Part model, mm, in its own coordinate system. Face numbers are marked on the shaded views. A direction names the side the tool comes from. Coordinates: 2 decimals unless noted, no trailing zeros. Write each loop counter-clockwise with the first axis right and the second up, starting at its lowest first coordinate (ties: lowest second). Pieces come first, ordered by that corner, then holes. Notation, with made-up numbers: (-7.5, 70) -> (22.5, 70) arc R26 cw to (22.5, 108) -> close; hole circle Ø5 at (-9.75, 38.25). An arc over 180 degrees is marked (long way). Write item = value, one per line.
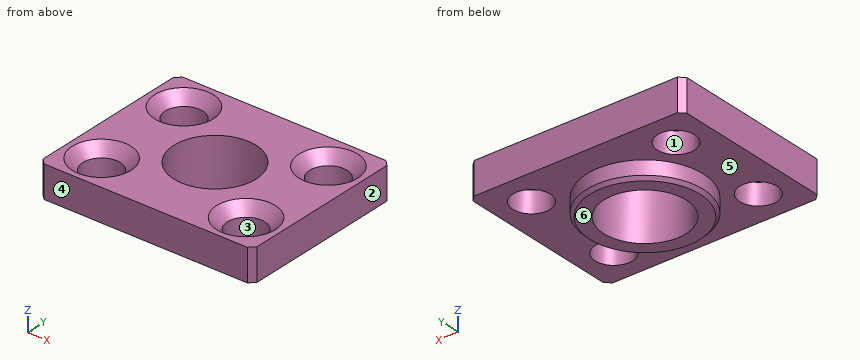
from build123d import *

# Parameters (mm, degrees)
SKETCH1_R           = 5.45
SKETCH1_R_2         = 3.85
BOSS_EXTRUDE1_DEPTH = 1.6
SKETCH2_W           = 20
SKETCH2_H           = 16
SKETCH2_R           = 3.85
SKETCH2_R_2         = 1.75
BOSS_EXTRUDE2_DEPTH = 3
CHAMFER1_SIZE       = 0.3
CHAMFER2_SIZE       = 1
CHAMFER3_SIZE       = 0.5


with BuildPart() as part:
    # Sketch1 → Boss-Extrude1 (new body)
    with BuildSketch(Plane.XY):
        Circle(SKETCH1_R)
        Circle(SKETCH1_R_2, mode=Mode.SUBTRACT)
    extrude(amount=BOSS_EXTRUDE1_DEPTH)

    # Sketch2 → Boss-Extrude2 (add)
    with BuildSketch(Plane.XY.offset(1.6)):
        Rectangle(SKETCH2_W, SKETCH2_H)
        Circle(SKETCH2_R, mode=Mode.SUBTRACT)
        with Locations((-6.75, 4.75)):
            Circle(SKETCH2_R_2, mode=Mode.SUBTRACT)
        with Locations((-6.75, -4.75)):
            Circle(SKETCH2_R_2, mode=Mode.SUBTRACT)
        with Locations((6.75, -4.75)):
            Circle(SKETCH2_R_2, mode=Mode.SUBTRACT)
        with Locations((6.75, 4.75)):
            Circle(SKETCH2_R_2, mode=Mode.SUBTRACT)
    extrude(amount=BOSS_EXTRUDE2_DEPTH)

    # Chamfer1
    chamfer1_edges = [part.edges().sort_by_distance(p)[0] for p in [
        (-5.45, 0, 0),
    ]]
    chamfer(chamfer1_edges, length=CHAMFER1_SIZE)

    # Chamfer2
    chamfer2_edges = [part.edges().sort_by_distance(p)[0] for p in [
        (-8.5, 4.75, 4.6),
        (-8.5, -4.75, 4.6),
        (5, -4.75, 4.6),
        (5, 4.75, 4.6),
    ]]
    chamfer(chamfer2_edges, length=CHAMFER2_SIZE)

    # Chamfer3
    chamfer3_edges = [part.edges().sort_by_distance(p)[0] for p in [
        (10, -8, 3.1),
        (10, 8, 3.1),
        (-10, 8, 3.1),
        (-10, -8, 3.1),
    ]]
    chamfer(chamfer3_edges, length=CHAMFER3_SIZE)


solid = part.part
Q1. Saw through at B-B on y = 0. Give the cut face in (x, z).
Model answer:
outline = (-10, 1.6) -> (-5.45, 1.6) -> (-5.45, 0.3) -> (-5.15, 0) -> (-3.85, 0) -> (-3.85, 4.6) -> (-10, 4.6) -> close; (3.85, 0) -> (5.15, 0) -> (5.45, 0.3) -> (5.45, 1.6) -> (10, 1.6) -> (10, 4.6) -> (3.85, 4.6) -> close
Q2. Saw through at D-D on z = 1.2. Give the cut face in (x, y), and give its area (3 significant figures).
Model answer:
outline = circle Ø10.9 at (0, 0); hole circle Ø7.7 at (0, 0)
area = 46.7 mm²
Q3. Pin check, flat tips, straight feed: pin 1 (5.5 mm diameter, centred on x = 6.75, y = -4.75, fed in from -Z); pin 2 (3 mm diameter, centred on x = -6.75, y = -4.75, fed in from -Z); pin 3 (4.5 mm diameter, centred on x = -6.75, y = 4.75, fed in from +Z); pin 4 (1 mm diameter, centred on x = -5, z = 1, fed in from -Y). Stop position of each tip, or through.
Model answer:
pin_1 = 1.6
pin_2 = through
pin_3 = 4.1
pin_4 = -3.07
Q4. Mould opens along X. For the marked faces 1, 2, 3 and 4 say: released by +X, released by -X, zero draft, split by the parting line, or undercut.
Model answer:
face_1 = undercut
face_2 = released by +X
face_3 = undercut
face_4 = zero draft
Q5. Saw through at C-C on z = 3. Give the cut face in (x, y), and give its area (3 significant figures).
Model answer:
outline = (-10, -7.5) -> (-9.5, -8) -> (9.5, -8) -> (10, -7.5) -> (10, 7.5) -> (9.5, 8) -> (-9.5, 8) -> (-10, 7.5) -> close; hole circle Ø3.5 at (-6.75, -4.75); hole circle Ø3.5 at (-6.75, 4.75); hole circle Ø7.7 at (0, 0); hole circle Ø3.5 at (6.75, -4.75); hole circle Ø3.5 at (6.75, 4.75)
area = 234 mm²
Q6. Probe line 1 (Y direction, x = 6.75, z = 2.1); line 2 (X direction, y = 6.25, z = 3.85); line 3 (Y direction, x = 0, z = 3.6). List the from-to ranges inside material, lowest first. Write a range as from..to.
Model answer:
line_1 = -8..-6.5, -3..3, 6.5..8
line_2 = -10..-8.07, -5.43..5.43, 8.07..10
line_3 = -8..-3.85, 3.85..8
Q7. Saw through at A-A on x = 0. Give the cut face in (y, z), and give its area (3 significant figures).
Model answer:
outline = (-8, 1.6) -> (-5.45, 1.6) -> (-5.45, 0.3) -> (-5.15, 0) -> (-3.85, 0) -> (-3.85, 4.6) -> (-8, 4.6) -> close; (3.85, 0) -> (5.15, 0) -> (5.45, 0.3) -> (5.45, 1.6) -> (8, 1.6) -> (8, 4.6) -> (3.85, 4.6) -> close
area = 29.9 mm²
Q8. Which spindle directions (+Z, -Z, +X, -X, +Y, -Y) get a long thin tool onto all of the face, cutting with end or side? Do the marked faces 5 and 6. Say none if no direction does.
Model answer:
face_5 = -Z
face_6 = -Z, +X, -X, +Y, -Y
